Source: CAD feature listing. Evaluate the final solid. Frame: model axes, mm. Face numbers are marked on the shaded views. A direction names the side the tool comes from. Give positions to 0.01 mm unless a question says otherwise; leave off trailing zeros. Order: outer loops, then holes, each group sorted by start corner. A loop starts at its lowest first (then second) coordinate and runs counter-clockwise, first axis right, second up.
from build123d import *

# Parameters (mm, degrees)
SKETCH2_R           = 12.5
BOSS_EXTRUDE1_DEPTH = 12
SKETCH6_R           = 12.5
BOSS_EXTRUDE2_DEPTH = 7.5
SKETCH5_R           = 1
CUT_EXTRUDE2_DEPTH  = 27.750389405
CUT_EXTRUDE3_START  = -15
SKETCH7_R           = 5.7225
CUT_EXTRUDE3_DEPTH  = 15


with BuildPart() as part:
    # Sketch1 → Revolve1 (revolve)
    with BuildSketch(Plane.XY, mode=Mode.PRIVATE) as revolve1_sk:
        with BuildLine():
            Line((0, 5.7225), (0, 7.2225))
            ThreePointArc((0, 7.2225), (3.667573597, 10.968130039), (8.5, 13))
            Line((8.5, 13), (8.5, 14.5))
            Line((8.5, 14.5), (20.5, 14.5))
            Line((20.5, 14.5), (20.5, 12.5))
            Line((20.5, 12.5), (22.5, 12.5))
            Line((22.5, 12.5), (22.5, 14.5))
            Line((22.5, 14.5), (30, 14.5))
            Line((30, 14.5), (30, 0))
            Line((30, 0), (15, 0))
            Line((15, 0), (15, 5.7225))
            Line((15, 5.7225), (0, 5.7225))
        make_face()
    revolve(revolve1_sk.sketch.rotate(Axis((0, 0, 0), (1, 0, 0)), 90), axis=Axis((0, 0, 0), (1, 0, 0)))

    # Sketch2 → Boss-Extrude1 (add)
    with BuildSketch(Plane(origin=(20.5, 0, 0), x_dir=(0, 0, -1), z_dir=(1, 0, 0))):
        Polygon((16.743157806, 0), (8.371578903, 14.5), (-8.371578903, 14.5), (-16.743157806, 0), (-8.371578903, -14.5), (8.371578903, -14.5), align=None)
        with Locations(Location((0, 0, 0), (0, 0, 180))):
            Circle(SKETCH2_R, mode=Mode.SUBTRACT)
    extrude(amount=-BOSS_EXTRUDE1_DEPTH)

    # Sketch6 → Boss-Extrude2 (add)
    with BuildSketch(Plane(origin=(30, 0, 0), x_dir=(0, 0, -1), z_dir=(1, 0, 0))):
        Polygon((16.743157806, 0), (8.371578903, 14.5), (-8.371578903, 14.5), (-16.743157806, 0), (-8.371578903, -14.5), (8.371578903, -14.5), align=None)
        with Locations(Location((0, 0, 0), (0, 0, 180))):
            Circle(SKETCH6_R, mode=Mode.SUBTRACT)
    extrude(amount=-BOSS_EXTRUDE2_DEPTH)

    # Sketch3 → Cut-Revolve1 (revolve, cut)
    with BuildSketch(Plane(origin=(0, 0, 0), x_dir=(1, 0, 0), z_dir=(0, 1, 0)), mode=Mode.PRIVATE) as cut_revolve1_sk:
        Polygon((18.256842194, 16.743157806), (20.5, 14.5), (20.5, 16.743157806), align=None)
        Polygon((24.743157806, 16.743157806), (22.5, 14.5), (22.5, 16.743157806), align=None)
        Polygon((8.5, 14.5), (10.743157806, 16.743157806), (8.5, 16.743157806), align=None)
        Polygon((27.756842194, 16.743157806), (30, 16.743157806), (30, 14.5), align=None)
    revolve(cut_revolve1_sk.sketch.rotate(Axis((0, 0, 0), (-1, 0, 0)), 270), axis=Axis((0, 0, 0), (-1, 0, 0)), mode=Mode.SUBTRACT)

    # Sketch5 → Cut-Extrude2 (cut, through all)
    with BuildSketch(Plane.ZY.offset(-15)):
        Circle(SKETCH5_R)
    extrude(amount=-CUT_EXTRUDE2_DEPTH, mode=Mode.SUBTRACT)

    # Sketch7 → Cut-Extrude3 (cut)
    with BuildSketch(Plane(origin=(30, 0, 0), x_dir=(0, 0, -1), z_dir=(1, 0, 0)).offset(CUT_EXTRUDE3_START)):
        with Locations(Location((0, 0, 0), (0, 0, 180))):
            Circle(SKETCH7_R)
    extrude(amount=CUT_EXTRUDE3_DEPTH, mode=Mode.SUBTRACT)


solid = part.part
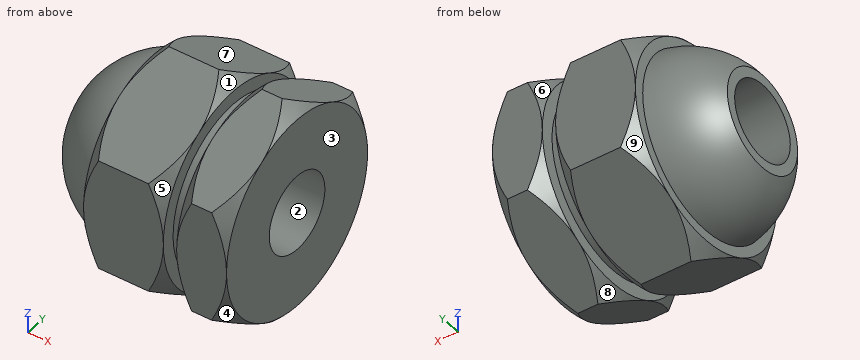
1) Ray query, L1, parallel to Y at x = 21, z = 0; L2, parallel to X at y = -10.25, z = 9; L3, parallel to Y at x = 15, z = -4. Return the intervals inside material, ascending.
Checks:
L1: y = -12.5 to -5.72, 5.72 to 12.5
L2: x = 8.5 to 20.5, 22.5 to 30
L3: y = -14.5 to -4.09, 4.09 to 14.5
2) Section query B-B on x = 7. Output: boundary loops of the cut face in (y, z) (1 decimal).
Checks:
outline: circle Ø25.2 at (0, 0); hole circle Ø11.4 at (0, 0)
3) Pull-direction query (Y, two-part tool) for the marked faces 1, 2, 3 and 4; classes: +Y half, -Y half, draft (parallel to the pull), parting line (faces both ways), or undercut.
Checks:
face 1: parting line
face 2: undercut
face 3: draft
face 4: -Y half
4) First-contact query: pin 1 Ø8 at (y, z) = (-7, 8) entering from -X; pin 2 Ø5 at (y, z) = (-10.5, -0.5) entering from -X; pin 3 Ø10 at (y, z) = (-11.5, 8) entering from -X; pin 4 Ø4 at (x, y) = (9, -2.5) entering from -Z. Flat tips, straight axial feed; report the tip coordinate or a pass-through.
Checks:
pin 1: stops at x = 0
pin 2: stops at x = 0.55
pin 3: stops at x = 1.39
pin 4: stops at z = -16.21
5) Reachability of the marked faces 5, 6, 7, 8 and 9 from +Z, -Z, +X, -X, +Y, -Y: full face, straight path, thin tool, end or side. Return the list, or none.
Checks:
face 5: +Z, -Y
face 6: +Z, +Y
face 7: +Z, +X, -X, +Y
face 8: -Z
face 9: -Z, -X, +Y
6) Section query A-A on x = 22. Output: boundary loops of the cut face in (y, z) (1 decimal).
Checks:
outline: circle Ø25 at (0, 0); hole circle Ø11.4 at (0, 0)
